from build123d import *

# Parameters (mm, degrees)
SKETCH_1_R      = 2
EXTRUDE_1_DEPTH = 6


with BuildPart() as part:
    # 草图1 → 凸台-拉伸1 (new body)
    with BuildSketch(Plane.XY):
        with BuildLine():
            Line((-119.735261546, 7.191323041), (120.264738454, 7.191323041))
            ThreePointArc((120.264738454, 7.191323041), (126.264738454, 1.191323041), (120.264738454, -4.808676959))
            Line((120.264738454, -4.808676959), (-119.735261546, -4.808676959))
            ThreePointArc((-119.735261546, -4.808676959), (-125.735261546, 1.191323041), (-119.735261546, 7.191323041))
        make_face()
        with Locations((-119.735261546, 1.191323041)):
            Circle(SKETCH_1_R, mode=Mode.SUBTRACT)
        with Locations((120.264738454, 1.191323041)):
            Circle(SKETCH_1_R, mode=Mode.SUBTRACT)
    extrude(amount=EXTRUDE_1_DEPTH)


solid = part.part
Check sheet for the modelled part. Datum: model origin and axes. Units: mm. Round coordinates to 2 decimals unless told otherwise and drop trailing zeros. Order: outer loops, then holes, each group sorted by start corner. A loop starts at its lowest first (then second) coordinate and runs counter-clockwise, first axis right, second up. Notation, with made-up numbers: M 59.5,53 L 78.5,53 A17 ccw 78.5,82 Z; hole C 24.25,73.5 d8. An arc over 180 degrees is marked long. One line per item, written item: value. Start each with the question number.
1. Gauge pin test, flat end, axial feed: P1, Ø1, axis at y = 2.5, z = 5, coming from the +X side. Record the tip position at first contact, or that the pin passes through.
2. Section check A-A on z = 4.25. Enter the section's corners in (x, y), and give its area (3 significant figures).
3. Release check for a two-part mould opening along X. For faces 1 (the cylindrical face through (118.79, 2.54, 2.96)), 2 (the cylindrical face through (126.263, 1.323, 2.958)), 3 (the flat face through (-1, 7.191, 3)) record: released by +X, released by -X, zero draft, split by the parting line, or undercut.
4. Scan lines: line 1 along X through (y, z) = (0.5, 2.8); line 2 along X through (y, z) = (0.25, 3.3); line 3 along X through (y, z) = (6.25, 0.7). Record each from-to range of solid material in increasing order.
Results found:
1. P1: x = 126.21
2. outline: M -119.74,-4.81 L 120.26,-4.81 A6 ccw 120.26,7.19 L -119.74,7.19 A6 ccw Z; hole C -119.74,1.19 d4; hole C 120.26,1.19 d4
2. area: 2,970 mm^2
3. face 1: undercut
3. face 2: released by +X
3. face 3: zero draft
4. line 1: -125.7 to -121.61, -117.86 to 118.39, 122.14 to 126.22
4. line 2: -125.66 to -121.5, -117.97 to 118.5, 122.03 to 126.19
4. line 3: -122.96 to 123.49
